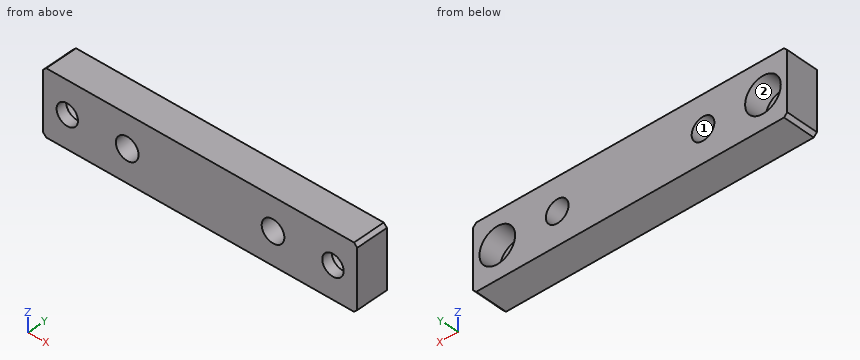
from build123d import *

# Parameters (mm, degrees)
SKETCH_1_W                   = 97
SKETCH_1_H                   = 20
EXTRUDE_1_DEPTH              = 5
M8X1_0_1_D                   = 7
HOLE_WIZARD_M6_1_D           = 6.6
HOLE_WIZARD_M6_1_CBORE_D     = 11
HOLE_WIZARD_M6_1_CBORE_DEPTH = 6.8
CHAMFER_1_SIZE               = 1


with BuildPart() as part:
    # 草图1 → 凸台-拉伸1 (new, symmetric)
    with BuildSketch(Plane(origin=(0, 0, 0), x_dir=(1, 0, 0), z_dir=(0, 1, 0))):
        Rectangle(SKETCH_1_W, SKETCH_1_H)
    extrude(amount=EXTRUDE_1_DEPTH, both=True)

    # M8x1.0 螺纹孔1 (through all)
    with Locations(Plane(origin=(0, 5, 0), x_dir=(1, 0, 0), z_dir=(0, 1, 0))):
        with Locations((-22.5, 0), (22.5, 0)):
            Hole(M8X1_0_1_D / 2)

    # M6 六角圆柱头螺钉的柱形沉头孔1 (through all)
    with Locations(Plane(origin=(0, 5, -3), x_dir=(-1, 0, 0), z_dir=(0, 1, 0))):
        with Locations((41, 3), (-41, 3)):
            CounterBoreHole(HOLE_WIZARD_M6_1_D / 2, HOLE_WIZARD_M6_1_CBORE_D / 2, HOLE_WIZARD_M6_1_CBORE_DEPTH)

    # 倒角1
    chamfer_1_edges = [part.edges().sort_by_distance(p)[0] for p in [
        (48.5, 0, 10),
        (-48.5, 0, 10),
        (-48.5, 0, -10),
        (48.5, 0, -10),
    ]]
    chamfer(chamfer_1_edges, length=CHAMFER_1_SIZE)


solid = part.part
Geometry: final body of the model. Coordinates: model frame, mm. Face numbers are marked on the shaded views. A direction names the side the tool comes from. Coordinates: 2 decimals unless noted, no trailing zeros. Write each loop counter-clockwise with the first axis right and the second up, starting at its lowest first coordinate (ties: lowest second). Pieces come first, ordered by that corner, then holes. Notation, with made-up numbers: (86, -27) - (139, -27) arc R20 cw to (139, 12) - close; hole circle Ø11 at (-14, -4.5). An arc over 180 degrees is marked (long way). Return JSON: item names as keys, results as strings.
Item 1: Section query A-A (x = -22.5). Output: boundary loops of the cut face in (y, z), and give its area (3 significant figures).
Completed:
{"outline": "(-5, -10) - (5, -10) - (5, -3.5) - (-5, -3.5) - close; (-5, 3.5) - (5, 3.5) - (5, 10) - (-5, 10) - close", "area": "130 mm2"}
Item 2: Pin query (flat end, axial travel): pin 1 Ø8 at (x, z) = (-22.5, 0) entering from -Y; pin 2 Ø10 at (x, z) = (-41, 0) entering from +Y. Return the tip coordinate at first contact, or that it passes through.
Completed:
{"pin 1": "stops at y = -5", "pin 2": "stops at y = -1.8"}
Item 3: Line query: L1, parallel to X at y = 1.75, z = -0.25; L2, parallel to X at y = -3, z = -2.25; L3, parallel to Z at x = -41, y = 0. Output: solid intervals per line, ascending.
Completed:
{"L1": "x = -48.5 to -46.49, -35.51 to -25.99, -19.01 to 19.01, 25.99 to 35.51, 46.49 to 48.5", "L2": "x = -48.5 to -43.41, -38.59 to -25.18, -19.82 to 19.82, 25.18 to 38.59, 43.41 to 48.5", "L3": "z = -10 to -5.5, 5.5 to 10"}
Item 4: Section query B-B (y = 1.75). Output: boundary loops of the cut face in (x, z), and give its area (3 significant figures).
Completed:
{"outline": "(-48.5, -9) - (-47.5, -10) - (47.5, -10) - (48.5, -9) - (48.5, 9) - (47.5, 10) - (-47.5, 10) - (-48.5, 9) - close; hole circle Ø11 at (-41, 0); hole circle Ø7 at (-22.5, 0); hole circle Ø7 at (22.5, 0); hole circle Ø11 at (41, 0)", "area": "1,670 mm2"}
Item 5: Reachability of the marked faces 1 and 2 from +Z, -Z, +X, -X, +Y, -Y: full face, straight path, thin tool, end or side. Return the list, or none.
Completed:
{"face 1": "+Y, -Y", "face 2": "+Y"}
Item 6: Section query D-D (x = -41). Output: boundary loops of the cut face in (y, z), and give its area (3 significant figures).
Completed:
{"outline": "(-5, -10) - (5, -10) - (5, -5.5) - (-1.8, -5.5) - (-1.8, -3.3) - (-5, -3.3) - close; (-5, 3.3) - (-1.8, 3.3) - (-1.8, 5.5) - (5, 5.5) - (5, 10) - (-5, 10) - close", "area": "104 mm2"}
Item 7: Section query C-C (z = -1.5). Output: boundary loops of the cut face in (x, y).
Completed:
{"outline": "(-48.5, -5) - (-43.94, -5) - (-43.94, -1.8) - (-46.29, -1.8) - (-46.29, 5) - (-48.5, 5) - close; (-38.06, -5) - (-25.66, -5) - (-25.66, 5) - (-35.71, 5) - (-35.71, -1.8) - (-38.06, -1.8) - close; (-19.34, -5) - (19.34, -5) - (19.34, 5) - (-19.34, 5) - close; (25.66, -5) - (38.06, -5) - (38.06, -1.8) - (35.71, -1.8) - (35.71, 5) - (25.66, 5) - close; (43.94, -5) - (48.5, -5) - (48.5, 5) - (46.29, 5) - (46.29, -1.8) - (43.94, -1.8) - close"}
